Geometry check sheet. Reference: the model listing, model coordinates, mm. Face numbers are marked on the shaded views. Round coordinates to 2 decimals unless told otherwise and drop trailing zeros. Write each loop counter-clockwise with the first axis right and the second up, starting at its lowest first coordinate (ties: lowest second). Pieces come first, ordered by that corner, then holes. Notation, with made-up numbers: (5.25, 86) - (18.25, 86) arc R26 cw to (18.25, 121) - close; hole circle Ø5 at (-3, 26.25). An arc over 180 degrees is marked (long way). Return JSON: item names as keys, results as strings.
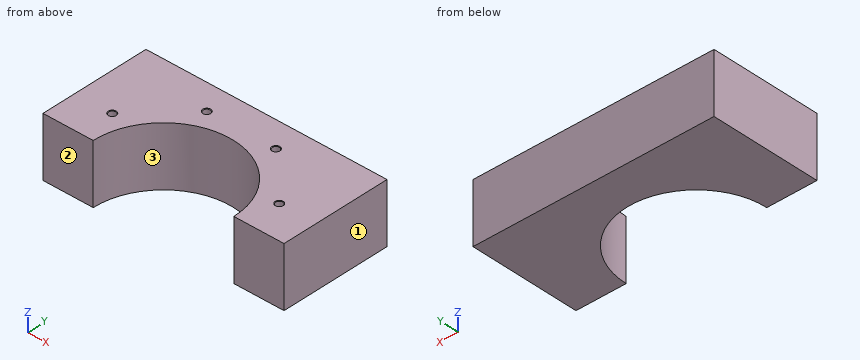
```python
from build123d import *

# Parameters (mm, degrees)
BOSS_EXTRUDE1_DEPTH          = 120
M16_TAPPED_HOLE1_D           = 14
M16_TAPPED_HOLE1_DEPTH       = 31.793975667
M16_TAPPED_HOLE1_CSINK_D     = 16.05
M16_TAPPED_HOLE1_CSINK_ANGLE = 90
M16_TAPPED_HOLE1_TIP         = 4.206024333


with BuildPart() as part:
    # Sketch1 → Boss-Extrude1 (new body)
    with BuildSketch(Plane.XY):
        with BuildLine():
            Line((-240, 220), (240, 220))
            Line((240, 220), (240, 0))
            Line((240, 0), (140, 0))
            ThreePointArc((140, 0), (0, 140), (-140, 0))
            Line((-140, 0), (-240, 0))
            Line((-240, 0), (-240, 220))
        make_face()
    extrude(amount=BOSS_EXTRUDE1_DEPTH)

    # M16 Tapped Hole1
    with Locations(Plane.XY.offset(120)):
        with Locations((-166.298315852, 68.883017826), (-68.883017826, 166.298315852), (68.883017826, 166.298315852), (166.298315852, 68.883017826)):
            CounterSinkHole(M16_TAPPED_HOLE1_D / 2, M16_TAPPED_HOLE1_CSINK_D / 2, depth=M16_TAPPED_HOLE1_DEPTH, counter_sink_angle=M16_TAPPED_HOLE1_CSINK_ANGLE)
            with Locations((0, 0, -(M16_TAPPED_HOLE1_DEPTH + M16_TAPPED_HOLE1_TIP / 2))):  # 118° drill point
                Cone(0, M16_TAPPED_HOLE1_D / 2, M16_TAPPED_HOLE1_TIP, mode=Mode.SUBTRACT)


solid = part.part
```
(1) Section check D-D, the plane x = 0. Enter the section's corners in (y, z), plus the area to 3 significant figures.
Response values:
{"outline": "(140, 0) - (220, 0) - (220, 120) - (140, 120) - close", "area": "9,600 mm^2"}
(2) Material ranges on line 1 along Y through (x, z) = (-72, 47); line 2 along Y through (x, z) = (0, 23.5); line 3 along X through (y, z) = (71, 56.5), recorded low to high. Write a range as [from, to].
Response values:
{"line 1": "y = [120.07, 220]", "line 2": "y = [140, 220]", "line 3": "x = [-240, -120.66], [120.66, 240]"}
(3) Section check B-B, the plane z = 70.5. Enter the section's corners in (x, y).
Response values:
{"outline": "(-240, 0) - (-140, 0) arc R140 cw to (140, 0) - (240, 0) - (240, 220) - (-240, 220) - close"}
(4) Release check for a two-part mould opening along X. For the marked faces 1, 2 and 3 record: pulls with the +X half, pulls with the -X half, needs draft (parallel to the pull), parting line crosses it, or undercut.
Response values:
{"face 1": "pulls with the +X half", "face 2": "needs draft", "face 3": "undercut"}
(5) Section check C-C, the plane z = 112. Enter the section's corners in (x, y), plus the area to 3 significant figures.
Response values:
{"outline": "(-240, 0) - (-140, 0) arc R140 cw to (140, 0) - (240, 0) - (240, 220) - (-240, 220) - close; hole circle Ø14 at (-166.3, 68.88); hole circle Ø14 at (-68.88, 166.3); hole circle Ø14 at (68.88, 166.3); hole circle Ø14 at (166.3, 68.88)", "area": "74,200 mm^2"}
(6) Gauge pin test, flat ends, axial feed: pin 1 (8 mm diameter, centred on x = 65, z = 58, fed in from -Y); pin 2 (12.5 mm diameter, centred on x = 166.3, y = 68.88, fed in from +Z). Record the tip position at first contact, or that the pin passes through.
Response values:
{"pin 1": "stops at y = 121.82", "pin 2": "stops at z = 87.76"}
(7) Section check A-A, the plane y = 102. Enter the section's corners in (x, z).
Response values:
{"outline": "(-240, 0) - (-95.9, 0) - (-95.9, 120) - (-240, 120) - close; (95.9, 0) - (240, 0) - (240, 120) - (95.9, 120) - close"}
